For this review, use the dimensioned drawing (mm, ordinates from the lowest corner) and the shaded views. A direction names the side the tool comes from. Give positions to 0.01 mm unless a question says otherwise; leave off trailing zeros. Write each loop counter-clockwise with the first axis right and the second up, starting at its lowest first coordinate (ties: lowest second). Pieces come first, ordered by that corner, then holes.
1) For P1, Ø5, axis at y = 2.5, z = 31, coming from the -X side; P2, Ø4, axis at y = 6.5, z = 19, coming from the -X side; P3, Ø1.5, axis at x = 3, z = 8, coming from the +Y side, all flat-tipped, find the tip position at first contact; note any pin that passes through.
2) Machinability: for the marked faces 1 and 2, which of the approach directions +Z, -Z, +X, -X, +Y, -Y give a long, thin tool a straight path to every point of the face, cutting with its end or side? Answer none if there is none.
3) Wall thickness on line 1 along Z through (x, y) = (8.75, 4.5); line 2 along Z through (x, y) = (7.75, 7) (1 decimal); line 3 along Y through (x, z) = (4, 30.5) (1 decimal): over which ranges is each line inside the solid? List them lowest first.
4) We need section B-B on y = 10.75. Give the boundary of the cut face in (x, z).
5) We need section D-D on y = 2.5. Give the boundary of the cut face in (x, z).
6) We need section C-C on z = 27.5. Give the boundary of the cut face in (x, y).
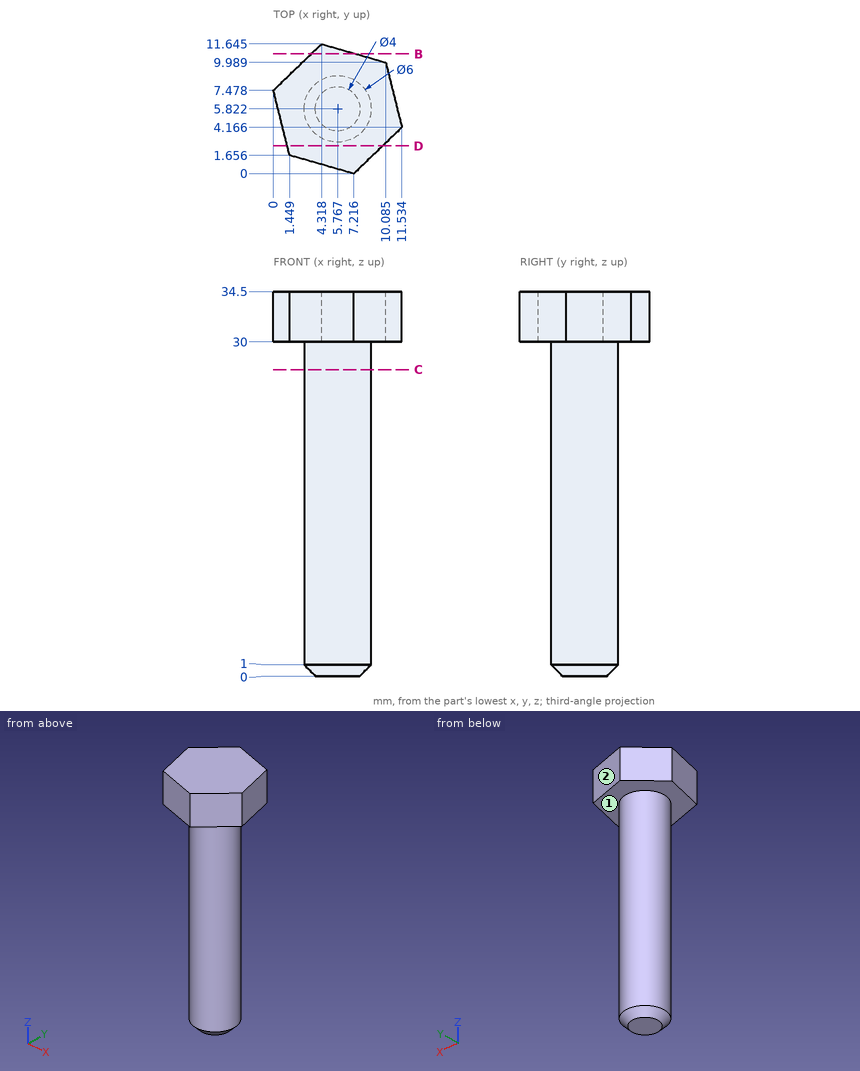
Results list:
1. P1: stops at x = 0.62
1. P2: stops at x = 2.77
1. P3: stops at y = 8.04
2. face 1: -Z
2. face 2: +Z, -Z, +X, +Y
3. line 1: z = 30 to 34.5
3. line 2: z = 0.3 to 34.5
3. line 3: y = 0.9 to 11.3
4. outline: (3.39, 30) - (7.43, 30) - (7.43, 34.5) - (3.39, 34.5) - close
5. outline: (1.24, 30) - (9.81, 30) - (9.81, 34.5) - (1.24, 34.5) - close
6. outline: circle Ø6 at (5.77, 5.82)
